```python
from build123d import *

# Parameters (mm, degrees)
SKETCH_1_W          = 290
SKETCH_1_H          = 150
EXTRUDE_1_DEPTH     = 350
SKETCH_2_R          = 7
EXTRUDE_2_DEPTH     = 5
SKETCH_3_W          = 145
SKETCH_3_H          = 23
CUT_EXTRUDE_1_DEPTH = 1
SKETCH_4_W          = 20
SKETCH_4_H          = 15
EXTRUDE_3_DEPTH     = 1.5
EXTRUDE_4_DEPTH     = 4.5
SKETCH_6_W          = 7
SKETCH_6_H          = 95
EXTRUDE_5_DEPTH     = 13


with BuildPart() as part:
    # 草图1 → 凸台-拉伸1 (new body)
    with BuildSketch(Plane(origin=(0, 0, 0), x_dir=(1, 0, 0), z_dir=(0, 1, 0))):
        Rectangle(SKETCH_1_W, SKETCH_1_H)
    extrude(amount=EXTRUDE_1_DEPTH)

    # 草图2 → 凸台-拉伸2 (add)
    with BuildSketch(Plane.XZ):
        with Locations(Location((-110, 63, 0), (0, 0, 90))):
            Circle(SKETCH_2_R)
        with Locations(Location((110, 63, 0), (0, 0, 90))):
            Circle(SKETCH_2_R)
        with Locations(Location((110, -67, 0), (0, 0, 90))):
            Circle(SKETCH_2_R)
        with Locations(Location((-110, -67, 0), (0, 0, 90))):
            Circle(SKETCH_2_R)
    extrude(amount=EXTRUDE_2_DEPTH)

    # 草图3 → 切除-拉伸1 (cut)
    with BuildSketch(Plane.ZY.offset(145)):
        with Locations((0, 160.5)):
            Rectangle(SKETCH_3_W, SKETCH_3_H)
    extrude(amount=-CUT_EXTRUDE_1_DEPTH, mode=Mode.SUBTRACT)

    # 草图4 → 凸台-拉伸3 (add)
    with BuildSketch(Plane.ZY.offset(144)):
        with Locations((-56.5, 160.5)):
            Rectangle(SKETCH_4_W, SKETCH_4_H)
    extrude(amount=EXTRUDE_3_DEPTH)

    # 草图5 → 凸台-拉伸4 (add, symmetric)
    with BuildSketch(Plane(origin=(0, 160.5, 0), x_dir=(-1, 0, 0), z_dir=(0, -1, 0))):
        with BuildLine():
            Line((145.5, 63.5), (149.5, 60.5))
            ThreePointArc((149.5, 60.5), (146.755035208, 55.270896288), (145.5, 49.5))
            Line((145.5, 49.5), (145.5, 63.5))
        make_face()
    extrude(amount=EXTRUDE_4_DEPTH, both=True)

    # 草图6 → 凸台-拉伸5 (add)
    with BuildSketch(Plane(origin=(145, 0, 0), x_dir=(0, 0, -1), z_dir=(1, 0, 0))):
        with Locations((26.5, 83.5)):
            Rectangle(SKETCH_6_W, SKETCH_6_H)
    extrude(amount=EXTRUDE_5_DEPTH)


solid = part.part
```
Source: CAD feature listing. Evaluate the final solid. Frame: model axes, mm. A direction names the side the tool comes from. Give positions to 0.01 mm unless a question says otherwise; leave off trailing zeros. Order: outer loops, then holes, each group sorted by start corner. A loop starts at its lowest first (then second) coordinate and runs counter-clockwise, first axis right, second up. Notation, with made-up numbers: (-38, 84.25) -> (-33, 84.25) arc R20 ccw to (-33, 99.25) -> close; hole circle Ø10 at (-9.5, 79). An arc over 180 degrees is marked (long way). Use a Markdown table: item, result.
Q1. Section A-A (z = 6.5). Return the cut outline in (x, y), and give its area (3 significant figures).
A:
| item | result |
|---|---|
| outline | (-145, 0) -> (145, 0) -> (145, 350) -> (-145, 350) -> (-145, 172) -> (-144, 172) -> (-144, 149) -> (-145, 149) -> close |
| area | 101,000 mm^2 |
Q2. Material intervals for line 1 (X direction, y = 50, z = 12.5); line 2 (Y direction, x = 17, z = 46); line 3 (X direction, y = 122, z = -27), sorted ascending. Write a range as [from, to].
A:
| item | result |
|---|---|
| line 1 | [-145, 145] |
| line 2 | [0, 350] |
| line 3 | [-145, 158] |
Q3. Section C-C (z = 63). Return the cut outline in (x, y).
A:
| item | result |
|---|---|
| outline | (-145, 0) -> (-117, 0) -> (-117, -5) -> (-103, -5) -> (-103, 0) -> (103, 0) -> (103, -5) -> (117, -5) -> (117, 0) -> (145, 0) -> (145, 350) -> (-145, 350) -> (-145, 172) -> (-144, 172) -> (-144, 149) -> (-145, 149) -> close |
Q4. Access query for faces 1 (the face through (151, 83, -23)), 2 (the face through (110, -5, 63)), 3 (the face through (-2, 173, -75)), 4 (the face through (151, 83, -30)), 5 (the face through (-116.94, -2.46, -67.91)). Directions: +Z, -Z, +X, -X, +Y, -Y. A direction counts if a zero-diameter tool reaches every point of the face in a straight line with its end or side. Return the directions, or none.
A:
| item | result |
|---|---|
| face 1 | +Z, +X, +Y, -Y |
| face 2 | +Z, -Z, +X, -X, -Y |
| face 3 | -Z, +X, -X, +Y, -Y |
| face 4 | -Z, +X, +Y, -Y |
| face 5 | -Y |
Q5. First-contact query: P1, Ø8, axis at x = -0.5, z = 15.5, coming from the -Y side; P2, Ø4.5, axis at x = -147.5, z = -53.5, coming from the -Y side; P3, Ø3.5, axis at x = 151, z = -27.5, coming from the +Y side. Flat tips, straight axial feed; report the tip coordinate or a pass-through.
A:
| item | result |
|---|---|
| P1 | y = 0 |
| P2 | y = 153 |
| P3 | y = 131 |
Q6. Section B-B (y = 72.5). Return the cut outline in (x, z), and give its area (3 significant figures).
A:
| item | result |
|---|---|
| outline | (-145, -75) -> (145, -75) -> (145, -30) -> (158, -30) -> (158, -23) -> (145, -23) -> (145, 75) -> (-145, 75) -> close |
| area | 43,600 mm^2 |
Q7. Section D-D (y = 227). Return the cut outline in (x, z).
A:
| item | result |
|---|---|
| outline | (-145, -75) -> (145, -75) -> (145, 75) -> (-145, 75) -> close |
Q8. Pull-direction query (X, two-part tool) for faces 6 (the face through (103.06, -2.46, -67.91)), 7 (the face through (-145, 173, 1)), 8 (the face through (-110, -5, 63)); classes: +X half, -X half, draft (parallel to the pull), parting line (faces both ways), or undercut.
A:
| item | result |
|---|---|
| face 6 | undercut |
| face 7 | -X half |
| face 8 | draft |
